The listing builds one solid part. Answer for the finished solid, in the listing's coordinates (mm). A direction names the side the tool comes from. Coordinates: 2 decimals unless noted, no trailing zeros. Write each loop counter-clockwise with the first axis right and the second up, starting at its lowest first coordinate (ties: lowest second). Pieces come first, ordered by that corner, then holes.
from build123d import *

# Parameters (mm, degrees)
BOSS_EXTRUDE1_DEPTH = 115


with BuildPart() as part:
    # Sketch1 → Boss-Extrude1 (new body)
    with BuildSketch(Plane.XY):
        with BuildLine():
            Line((-4.5, 5.5), (-4.5, 5.04))
            ThreePointArc((-4.5, 5.04), (-3.46, 4), (-4.5, 2.96))
            Line((-4.5, 2.96), (-4.5, 0.296984848))
            Line((-4.5, 0.296984848), (-4.203015152, 0))
            Line((-4.203015152, 0), (4.203015152, 0))
            Line((4.203015152, 0), (4.5, 0.296984848))
            Line((4.5, 0.296984848), (4.5, 2.96))
            ThreePointArc((4.5, 2.96), (3.46, 4), (4.5, 5.04))
            Line((4.5, 5.04), (4.5, 5.5))
            Line((4.5, 5.5), (-4.5, 5.5))
        make_face()
    extrude(amount=BOSS_EXTRUDE1_DEPTH)

    # Sketch2 → Cut-Revolve1 (revolve, cut)
    with BuildSketch(Plane(origin=(0, 0, 0), x_dir=(0, 0, -1), z_dir=(1, 0, 0)), mode=Mode.PRIVATE) as cut_revolve1_sk:
        Polygon((-7.5, 5.5), (-4.5, 5.5), (-4.5, 2), (-5.75, 2), (-5.75, 0), (-7.5, 0), align=None)
    revolve(cut_revolve1_sk.sketch.rotate(Axis((0, 0, 7.5), (0, 1, 0)), 180), axis=Axis((0, 0, 7.5), (0, 1, 0)), mode=Mode.SUBTRACT)

    # Sketch3 → Cut-Revolve2 (revolve, cut)
    with BuildSketch(Plane(origin=(0, 0, 0), x_dir=(0, 0, -1), z_dir=(1, 0, 0)), mode=Mode.PRIVATE) as cut_revolve2_sk:
        Polygon((-107.5, 5.5), (-104.5, 5.5), (-104.5, 2), (-105.75, 2), (-105.75, 0), (-107.5, 0), align=None)
    revolve(cut_revolve2_sk.sketch.rotate(Axis((0, 0, 107.5), (0, 1, 0)), 180), axis=Axis((0, 0, 107.5), (0, 1, 0)), mode=Mode.SUBTRACT)

    # Sketch4 → Cut-Revolve3 (revolve, cut)
    with BuildSketch(Plane(origin=(0, 0, 0), x_dir=(0, 0, -1), z_dir=(1, 0, 0)), mode=Mode.PRIVATE) as cut_revolve3_sk:
        Polygon((-87.5, 5.5), (-84.5, 5.5), (-84.5, 2), (-85.75, 2), (-85.75, 0), (-87.5, 0), align=None)
    revolve(cut_revolve3_sk.sketch.rotate(Axis((0, 0, 87.5), (0, 1, 0)), 180), axis=Axis((0, 0, 87.5), (0, 1, 0)), mode=Mode.SUBTRACT)

    # Sketch5 → Cut-Revolve4 (revolve, cut)
    with BuildSketch(Plane(origin=(0, 0, 0), x_dir=(0, 0, -1), z_dir=(1, 0, 0)), mode=Mode.PRIVATE) as cut_revolve4_sk:
        Polygon((-67.5, 5.5), (-64.5, 5.5), (-64.5, 2), (-65.75, 2), (-65.75, 0), (-67.5, 0), align=None)
    revolve(cut_revolve4_sk.sketch.rotate(Axis((0, 0, 67.5), (0, 1, 0)), 180), axis=Axis((0, 0, 67.5), (0, 1, 0)), mode=Mode.SUBTRACT)

    # Sketch6 → Cut-Revolve5 (revolve, cut)
    with BuildSketch(Plane(origin=(0, 0, 0), x_dir=(0, 0, -1), z_dir=(1, 0, 0)), mode=Mode.PRIVATE) as cut_revolve5_sk:
        Polygon((-47.5, 5.5), (-44.5, 5.5), (-44.5, 2), (-45.75, 2), (-45.75, 0), (-47.5, 0), align=None)
    revolve(cut_revolve5_sk.sketch.rotate(Axis((0, 0, 47.5), (0, 1, 0)), 180), axis=Axis((0, 0, 47.5), (0, 1, 0)), mode=Mode.SUBTRACT)

    # Sketch7 → Cut-Revolve6 (revolve, cut)
    with BuildSketch(Plane(origin=(0, 0, 0), x_dir=(0, 0, -1), z_dir=(1, 0, 0)), mode=Mode.PRIVATE) as cut_revolve6_sk:
        Polygon((-27.5, 5.5), (-24.5, 5.5), (-24.5, 2), (-25.75, 2), (-25.75, 0), (-27.5, 0), align=None)
    revolve(cut_revolve6_sk.sketch.rotate(Axis((0, 0, 27.5), (0, 1, 0)), 180), axis=Axis((0, 0, 27.5), (0, 1, 0)), mode=Mode.SUBTRACT)


solid = part.part
Q1. Which of the six approach directions +Z, -Z, +X, -X, +Y, -Y give full straight-line access (tool end or side, diameter ignored) to faces 1 (the face through (0.1, 3.7, 24.5)), 2 (the face through (-0.67, 0.986, 49.117))?
Answers below:
face 1: +Y
face 2: +Y, -Y
Q2. Determine the mould class of faces 3 (the face through (0.526, 0.986, 9.169)), 4 (the face through (-1.8, 3.7, 65.1)), 5 (the face through (0, 3, 0)), 6 (the face through (-4.5, 2, 57)) for opening direction Z: released by +Z, released by -Z, zero draft, split by the parting line, or undercut.
Answers below:
face 3: undercut
face 4: undercut
face 5: released by -Z
face 6: zero draft
Q3. Given pin 1 (1.8 mm diameter, centred on x = 0.5, z = 68, fed in from +Y) (3 decimals); pin 2 (4.5 mm diameter, centred on x = 0, z = 107.5, fed in from +Y); pin 3 (5 mm diameter, centred on x = -1, z = 47, fed in from +Y), each flat-ended and moving along its own axis, determine where each tip first touches the part or whether it passes through.
Answers below:
pin 1: passes through
pin 2: stops at y = 2
pin 3: stops at y = 5.5
Q4. The part is cut by section B-B, the plane y = 4. Write down the section's boundary in (x, z).
Answers below:
outline: (-3.46, 0) - (3.46, 0) - (3.46, 115) - (-3.46, 115) - close; hole circle Ø6 at (0, 7.5); hole circle Ø6 at (0, 27.5); hole circle Ø6 at (0, 47.5); hole circle Ø6 at (0, 67.5); hole circle Ø6 at (0, 87.5); hole circle Ø6 at (0, 107.5)
Q5. Find the intervals of material crossed by probe 1 along X at (y, z) = (0.75, 47.5); probe 2 along X at (y, z) = (3.1, 87.5); probe 3 along Y at (x, z) = (-2, 88), in increasing order.
Answers below:
probe 1: x = -4.5 to -1.75, 1.75 to 4.5
probe 2: x = -3.98 to -3, 3 to 3.98
probe 3: y = 0 to 2
Q6. The part is cut by section A-A, the plane z = 107.5. Write down the section's boundary in (x, y), then the cut area to 3 significant figures.
Answers below:
outline: (-4.5, 0.3) - (-4.2, 0) - (-1.75, 0) - (-1.75, 2) - (-3, 2) - (-3, 5.5) - (-4.5, 5.5) - (-4.5, 5.04) arc R1.04 cw to (-4.5, 2.96) - close; (1.75, 0) - (4.2, 0) - (4.5, 0.3) - (4.5, 2.96) arc R1.04 cw to (4.5, 5.04) - (4.5, 5.5) - (3, 5.5) - (3, 2) - (1.75, 2) - close
area: 18.0 mm2
Q7. The part is cut by section C-C, the plane z = 73. Write down the section's boundary in (x, y), then the cut area to 3 significant figures.
Answers below:
outline: (-4.5, 0.3) - (-4.2, 0) - (4.2, 0) - (4.5, 0.3) - (4.5, 2.96) arc R1.04 cw to (4.5, 5.04) - (4.5, 5.5) - (-4.5, 5.5) - (-4.5, 5.04) arc R1.04 cw to (-4.5, 2.96) - close
area: 46.0 mm2
